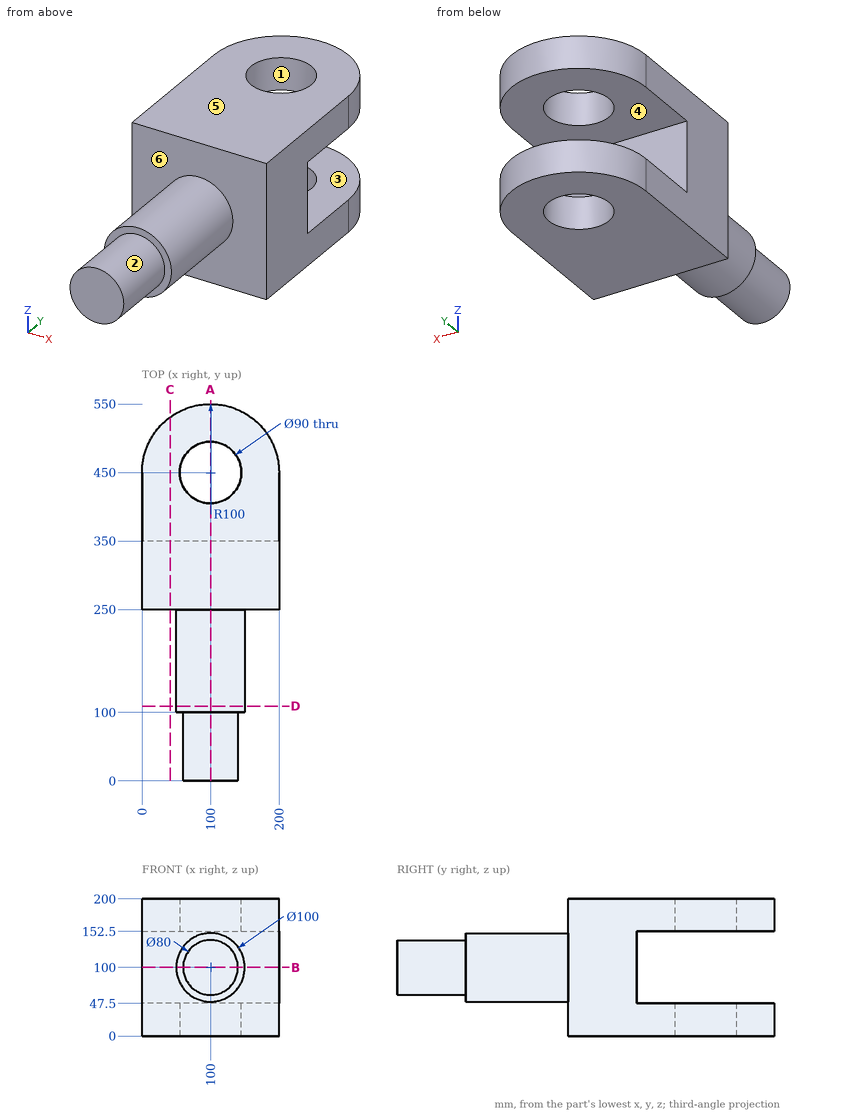
The figure shows three views and two pictorial views of one solid part (mm, origin at its lowest corner). Answer the questions. A direction names the side the tool comes from. Give positions to 0.01 mm unless a question says otherwise; leave off trailing zeros. Order: outer loops, then holes, each group sorted by start corner. A loop starts at its lowest first (then second) coordinate and runs counter-clockwise, first axis right, second up. Notation, with made-up numbers: M 13.25,-15.5 L 65.25,-15.5 A28 ccw 65.25,7.5 Z; hole C 46,18 d11. An arc over 180 degrees is marked long. Return JSON: item names as keys, results as strings.
Q1. Find section C-C, the plane x = 41. Write down the section's boundary in (y, z), and give its area (3 significant figures).
Answer below:
{"outline": "M 250,0 L 530.74,0 L 530.74,47.5 L 350,47.5 L 350,152.5 L 530.74,152.5 L 530.74,200 L 250,200 Z", "area": "37,200 mm^2"}
Q2. Each of these flat-tipped pins is pushed along its axis until it touches: pin 1 (3 mm diameter, centred on x = 34.5, z = 169, fed in from +Y); pin 2 (10 mm diameter, centred on x = 160.5, z = 77.5, fed in from +Y); pin 3 (5 mm diameter, centred on y = 214, z = 138.5, fed in from +X); pin 4 (6 mm diameter, centred on y = 325.5, z = 140.5, fed in from -X). Where does it stop, or does it pass through?
Answer below:
{"pin 1": "stops at y = 526.84", "pin 2": "stops at y = 350", "pin 3": "stops at x = 134.7", "pin 4": "stops at x = 0"}
Q3. Find section B-B, the plane z = 100. Write down the section's boundary in (x, y).
Answer below:
{"outline": "M 0,250 L 50,250 L 50,100 L 60,100 L 60,0 L 140,0 L 140,100 L 150,100 L 150,250 L 200,250 L 200,350 L 0,350 Z"}
Q4. Find the intervals of material crossed by line 1 along X through (y, z) = (450, 170); line 2 along Y through (x, z) = (100, 25); line 3 along Z through (x, y) = (188.5, 431), in increasing order. Write a range as [from, to].
Answer below:
{"line 1": "x = [0, 55], [145, 200]", "line 2": "y = [250, 405], [495, 550]", "line 3": "z = [0, 47.5], [152.5, 200]"}
Q5. The mould has two halves that part along Z. Classify the marked faces 1, 2 and 3: pulls with the +Z half, pulls with the -Z half, needs draft (parallel to the pull), parting line crosses it, or undercut.
Answer below:
{"face 1": "needs draft", "face 2": "parting line crosses it", "face 3": "undercut"}
Q6. Find section A-A, the plane x = 100. Write down the section's boundary in (y, z), and give its area (4 significant figures).
Answer below:
{"outline": "M 0,60 L 100,60 L 100,50 L 250,50 L 250,0 L 405,0 L 405,47.5 L 350,47.5 L 350,152.5 L 405,152.5 L 405,200 L 250,200 L 250,150 L 100,150 L 100,140 L 0,140 Z; M 495,0 L 550,0 L 550,47.5 L 495,47.5 Z; M 495,152.5 L 550,152.5 L 550,200 L 495,200 Z", "area": "53,450 mm^2"}
Q7. Find section D-D, the plane y = 109. Write down the section's boundary in (x, z).
Answer below:
{"outline": "C 100,100 d100"}
Q8. Which of the six approach directions +Z, -Z, +X, -X, +Y, -Y give full straight-line access (tool end or side, diameter ignored) to the marked faces 4, 5 and 6?
Answer below:
{"face 4": "+X, -X, +Y", "face 5": "+Z, +X, -X, +Y, -Y", "face 6": "-Y"}
